```python
from build123d import *

# Parameters (mm, degrees)
SKETCH_1_R          = 20
EXTRUDE_1_DEPTH     = 40
SKETCH_2_R          = 4
CUT_EXTRUDE_1_DEPTH = 49.989794856
SKETCH_3_R          = 7
CUT_EXTRUDE_2_DEPTH = 28
CUT_EXTRUDE_3_DEPTH = 13
CUT_EXTRUDE_START   = -13
CUT_EXTRUDE_4_DEPTH = 13


with BuildPart() as part:
    # 草图1 → 凸台-拉伸1 (new body)
    with BuildSketch(Plane.XY):
        Circle(SKETCH_1_R)
    extrude(amount=EXTRUDE_1_DEPTH)

    # 草图2 → 切除-拉伸1 (cut, through all)
    with BuildSketch(Plane.XY.offset(40)):
        Circle(SKETCH_2_R)
    extrude(amount=-CUT_EXTRUDE_1_DEPTH, mode=Mode.SUBTRACT)

    # 草图3 → 切除-拉伸2 (cut)
    with BuildSketch(Plane.XY.offset(40)):
        Circle(SKETCH_3_R)
    extrude(amount=-CUT_EXTRUDE_2_DEPTH, mode=Mode.SUBTRACT)

    # 草图4 → 切除-拉伸3 (cut)
    with BuildSketch(Plane.XY.offset(40)):
        with BuildLine():
            Line((17.228226516, -1.3), (17.228226516, 1.3))
            Line((17.228226516, 1.3), (6.878226516, 1.3))
            ThreePointArc((6.878226516, 1.3), (7, 0), (6.878226516, -1.3))
            Line((6.878226516, -1.3), (17.228226516, -1.3))
        make_face()
    extrude(amount=-CUT_EXTRUDE_3_DEPTH, mode=Mode.SUBTRACT)

    # 草图5 → 切除-拉伸4 (cut)
    with BuildSketch(Plane(origin=(0, 0, 0), x_dir=(-1, 0, 0), z_dir=(0, 0, -1)).offset(CUT_EXTRUDE_START)):
        with BuildLine():
            Line((16.948468057, -0.64), (16.948468057, 0.64))
            Line((16.948468057, 0.64), (3.948468057, 0.64))
            ThreePointArc((3.948468057, 0.64), (4, 0), (3.948468057, -0.64))
            Line((3.948468057, -0.64), (16.948468057, -0.64))
        make_face()
    extrude(amount=CUT_EXTRUDE_4_DEPTH, mode=Mode.SUBTRACT)


solid = part.part
```
For this review, take the finished solid that the model builds, in its own axes (mm). A direction names the side the tool comes from. Coordinates: 2 decimals unless noted, no trailing zeros. Order: outer loops, then holes, each group sorted by start corner. A loop starts at its lowest first (then second) coordinate and runs counter-clockwise, first axis right, second up. Notation, with made-up numbers: (1, 9) -> (18, 9) arc R36 cw to (18, 44) -> close; hole circle Ø9 at (82, 38.5). An arc over 180 degrees is marked (long way). Use CSV: the item, a comma, the result in double quotes. Start each with the question number.
Item 1: Wall thickness on probe 1 along Y at (x, z) = (0, 7.5); probe 2 along Y at (x, z) = (0, 26); probe 3 along Z at (x, y) = (2, 5): over which ranges is each line inside the solid? List them lowest first.
Item 2: We need section D-D, the plane y = -6. Give the boundary of the cut face in (x, z).
Item 3: We need section A-A, the plane y = 0. Give the boundary of the cut face in (x, z).
Item 4: For faces 1 (the face through (-11, 0.64, 7)), 2 (the face through (4, 0, 6)), 3 (the face through (12, 1.3, 34)), list the 3-axis set-ups (+Z, -Z, +X, -X, +Y, -Y) from which the entire face can be reached by the end or side of a thin tool; tool diameter is ignored.
Item 5: We need section B-B, the plane x = 0. Give the boundary of the cut face in (y, z), then the cut area to 3 significant figures.
Item 6: We need section C-C, the plane z = 7.5. Give the boundary of the cut face in (x, y), then the cut area to 3 significant figures.
Item 7: Insertion check: pin 1 (8.5 mm diameter, centred on x = 13.5, z = 32, fed in from -Y); pin 2 (5 mm diameter, centred on x = 13, z = 36.5, fed in from +Y); pin 3 (2 mm diameter, centred on x = -6, z = 19, fed in from +Y); pin 4 (5 mm diameter, centred on x = 0, y = 0, fed in from -Z). Each pin has a flat end and moves straight along its axis. Give the tip position at first contact, or say it passes through.
Item 8: Draft analysis for pull direction Y (two halves, no side actions). For faces 4 (the face through (0, -9, 40)), 5 (the face through (6.677, 2.103, 26.196)), 6 (the face through (-4.336, -19.524, 19.72)), state which applies: pulls with the +Y half, pulls with the -Y half, needs draft (parallel to the pull), parting line crosses it, or undercut.
Derived:
1,probe 1,"y = -20 to -4, 4 to 20"
1,probe 2,"y = -20 to -7, 7 to 20"
1,probe 3,"z = 0 to 12"
2,outline,"(-19.08, 0) -> (19.08, 0) -> (19.08, 40) -> (3.61, 40) -> (3.61, 12) -> (-3.61, 12) -> (-3.61, 40) -> (-19.08, 40) -> close"
3,outline,"(-20, 0) -> (-16.95, 0) -> (-16.95, 13) -> (-7, 13) -> (-7, 40) -> (-20, 40) -> close; (4, 0) -> (20, 0) -> (20, 40) -> (17.23, 40) -> (17.23, 27) -> (7, 27) -> (7, 12) -> (4, 12) -> close"
4,face 1,"-Z"
4,face 2,"+Z, -Z"
4,face 3,"+Z"
5,outline,"(-20, 0) -> (-4, 0) -> (-4, 12) -> (-7, 12) -> (-7, 40) -> (-20, 40) -> close; (4, 0) -> (20, 0) -> (20, 40) -> (7, 40) -> (7, 12) -> (4, 12) -> close"
5,area,"1,110 mm^2"
6,outline,"circle Ø40 at (0, 0); hole (-16.95, -0.64) -> (-3.95, -0.64) arc R4 ccw (long way) to (-3.95, 0.64) -> (-16.95, 0.64) -> close"
6,area,"1,190 mm^2"
7,pin 1,"stops at y = -17.73"
7,pin 2,"stops at y = 17.02"
7,pin 3,"stops at y = 19.36"
7,pin 4,"passes through"
8,face 4,"needs draft"
8,face 5,"undercut"
8,face 6,"parting line crosses it"
